from build123d import *

# Parameters (mm, degrees)
SKETCH_1_W          = 150
SKETCH_1_H          = 100
EXTRUDE_1_DEPTH     = 30
SKETCH_2_R          = 31.5
SKETCH_2_R_2        = 16
EXTRUDE_2_DEPTH     = 10
SKETCH_3_R          = 16
CUT_EXTRUDE_1_DEPTH = 96
SKETCH_4_R          = 6
CUT_EXTRUDE_2_DEPTH = 99.615414617


with BuildPart() as part:
    # 草图1 → 凸台-拉伸1 (new body)
    with BuildSketch(Plane.XY):
        Rectangle(SKETCH_1_W, SKETCH_1_H)
    extrude(amount=EXTRUDE_1_DEPTH)

    # 草图2 → 凸台-拉伸2 (add)
    with BuildSketch(Plane.XY.offset(30)):
        with Locations(Location((0, 0, 0), (0, 0, 180))):
            Circle(SKETCH_2_R)
        Circle(SKETCH_2_R_2, mode=Mode.SUBTRACT)
    extrude(amount=EXTRUDE_2_DEPTH)

    # 草图3 → 切除-拉伸1 (cut, through all)
    with BuildSketch(Plane.XY.offset(30)):
        Circle(SKETCH_3_R)
    extrude(amount=-CUT_EXTRUDE_1_DEPTH, mode=Mode.SUBTRACT)

    # 草图4 → 切除-拉伸2 (cut, through all)
    with BuildSketch(Plane(origin=(0, 0, 0), x_dir=(-1, 0, 0), z_dir=(0, 0, -1))):
        with Locations((-58.5, 30)):
            Circle(SKETCH_4_R)
        with Locations((48.5, 30)):
            Circle(SKETCH_4_R)
        with Locations((48.5, -30)):
            Circle(SKETCH_4_R)
        with Locations((-58.5, -30)):
            Circle(SKETCH_4_R)
    extrude(amount=-CUT_EXTRUDE_2_DEPTH, mode=Mode.SUBTRACT)


solid = part.part
Verification items for the finished model (mm, model axes). Give positions to 0.01 mm unless a question says otherwise; leave off trailing zeros. Loops run counter-clockwise (first coordinate to the right, second up) from the corner with the lowest first, then second, coordinate; pieces in that order, holes last.
1. Cross-section at D-D on x = 0. Record the cut outline in (y, z), and give its area (3 significant figures).
Derived:
outline: (-50, 0) - (-16, 0) - (-16, 40) - (-31.5, 40) - (-31.5, 30) - (-50, 30) - close; (16, 0) - (50, 0) - (50, 30) - (31.5, 30) - (31.5, 40) - (16, 40) - close
area: 2,350 mm2
2. Cross-section at B-B on y = 0. Record the cut outline in (x, z), and give its area (3 significant figures).
Derived:
outline: (-75, 0) - (-16, 0) - (-16, 40) - (-31.5, 40) - (-31.5, 30) - (-75, 30) - close; (16, 0) - (75, 0) - (75, 30) - (31.5, 30) - (31.5, 40) - (16, 40) - close
area: 3,850 mm2
3. Go/stop test with a flat-tipped pin: P1, Ø19, axis at x = -48.5, y = -30, coming from the +Z side. Record where the tip stops, or that it passes through.
Derived:
P1: stops at z = 30
4. Release check for a two-part mould opening along Y. For faces 1 (the flat face through (-18, 1, 0)), 2 (the cylindrical face through (63.26, 26.35, 14.79)), 3 (the cylindrical face through (4.101, -31.232, 34.93)) record: +Y half, -Y half, draft (parallel to the pull), parting line (faces both ways), or undercut.
Derived:
face 1: draft
face 2: undercut
face 3: parting line
5. Cross-section at C-C on z = 14.5. Record the cut outline in (x, y).
Derived:
outline: (-75, -50) - (75, -50) - (75, 50) - (-75, 50) - close; hole circle Ø12 at (-48.5, -30); hole circle Ø12 at (-48.5, 30); hole circle Ø32 at (0, 0); hole circle Ø12 at (58.5, -30); hole circle Ø12 at (58.5, 30)
6. Material ranges on probe 1 along Y at (x, z) = (58.5, 18); probe 2 along Y at (x, z) = (60, 9); probe 3 along Z at (x, y) = (20, -27), recorded low to high.
Derived:
probe 1: y = -50 to -36, -24 to 24, 36 to 50
probe 2: y = -50 to -35.81, -24.19 to 24.19, 35.81 to 50
probe 3: z = 0 to 30
7. Cross-section at A-A on x = 58.5. Record the cut outline in (y, z), and give its area (3 significant figures).
Derived:
outline: (-50, 0) - (-36, 0) - (-36, 30) - (-50, 30) - close; (-24, 0) - (24, 0) - (24, 30) - (-24, 30) - close; (36, 0) - (50, 0) - (50, 30) - (36, 30) - close
area: 2,280 mm2
